```python
from build123d import *

# Parameters (mm, degrees)
BOSS_EXTRUDE1_DEPTH = 10


with BuildPart() as part:
    # Sketch1 → Boss-Extrude1 (new body)
    with BuildSketch(Plane.XY):
        Polygon((0, 0), (0, 280), (20, 280), (180, 20), (180, 0), align=None)
    extrude(amount=BOSS_EXTRUDE1_DEPTH)


solid = part.part
```
Verification items for the finished model (mm, model axes). Coordinates: 2 decimals unless noted, no trailing zeros. Order: outer loops, then holes, each group sorted by start corner. A loop starts at its lowest first (then second) coordinate and runs counter-clockwise, first axis right, second up. Notation, with made-up numbers: (-38.5, 57.5) -> (20.5, 57.5) arc R33 cw to (20.5, 85.5) -> close; hole circle Ø5 at (-37.75, 65.5). An arc over 180 degrees is marked (long way). Put each result on its own line as item: value. Start each with the question number.
1) Go/stop test with a flat-tipped pin: pin 1 (12 mm diameter, centred on x = 82, y = 202, fed in from +Z). Record where the tip stops, or that it passes through.
2) Material ranges on L1, parallel to Y at x = 38, z = 3.75; L2, parallel to Y at x = 79.5, z = 6.5; L3, parallel to X at y = 198.5, z = 3, recorded low to high.
3) Cross-section at B-B (x = 156). Enter the section's corners in (y, z).
4) Cross-section at A-A (z = 3.75). Enter the section's corners in (x, y), plus the area to 3 significant figures.
5) Cross-section at C-C (y = 189). Enter the section's corners in (x, z), plus the area to 3 significant figures.
Geometry check:
1. pin 1: passes through
2. L1: y = 0 to 250.75
2. L2: y = 0 to 183.31
2. L3: x = 0 to 70.15
3. outline: (0, 0) -> (59, 0) -> (59, 10) -> (0, 10) -> close
4. outline: (0, 0) -> (180, 0) -> (180, 20) -> (20, 280) -> (0, 280) -> close
4. area: 29,600 mm^2
5. outline: (0, 0) -> (76, 0) -> (76, 10) -> (0, 10) -> close
5. area: 760 mm^2
